For this review, take the finished solid that the model builds, in its own axes (mm). Give positions to 0.01 mm unless a question says otherwise; leave off trailing zeros. Write each loop counter-clockwise with the first axis right and the second up, starting at its lowest first coordinate (ties: lowest second). Pieces come first, ordered by that corner, then holes. Notation, with made-up numbers: M 48,-26 L 99,-26 A14 cw 99,-18 Z; hole C 5,84 d8. An arc over 180 degrees is marked long. Write item = value, one per line.
```python
from build123d import *

# Parameters (mm, degrees)
SKETCH1_R                  = 11.25
BOSS_EXTRUDE1_DEPTH        = 2.5
SKETCH2_R                  = 1.6
CUT_EXTRUDE1_DEPTH         = 2.5
M3_TAPPED_HOLE1_AT_2_COUNT = 2
M3_TAPPED_HOLE1_AT_2_PITCH = 32.526911935
CHAMFER1_SIZE              = 0.3


with BuildPart() as part:
    # Sketch1 → Boss-Extrude1 (new body)
    with BuildSketch(Plane.XY):
        Polygon((-14, -12.5), (-12.5, -14), (12.5, -14), (14, -12.5), (14, 12.5), (12.5, 14), (-12.5, 14), (-14, 12.5), align=None)
        Circle(SKETCH1_R, mode=Mode.SUBTRACT)
    extrude(amount=BOSS_EXTRUDE1_DEPTH)

    # Sketch2 → Cut-Extrude1 (cut)
    with BuildSketch(Plane.XY.offset(2.5)):
        with Locations((-11.5, 11.5)):
            Circle(SKETCH2_R)
        with Locations((11.5, -11.5)):
            Circle(SKETCH2_R)
    extrude(amount=-CUT_EXTRUDE1_DEPTH, mode=Mode.SUBTRACT)

    # Sketch4 → M3 Tapped Hole1 (revolve, cut)
    with BuildSketch(Plane(origin=(-11.5, -11.5, 2.5), x_dir=(0, -1, 0), z_dir=(1, 0, 0))):
        Polygon((0, 0), (0, 2.5), (1.6, 2.5), (1.25, 2.15), (1.25, 0.35), (1.6, 0), align=None)
    m3_tapped_hole1 = revolve(axis=Axis((-11.5, -11.5, 8.85), (0, 0, -1)), mode=Mode.SUBTRACT)

    # M3 Tapped Hole1 at 2: M3 Tapped Hole1 ×2
    with Locations(*[Vector(0.7071067811865476, 0.7071067811865476, 0) * (i * M3_TAPPED_HOLE1_AT_2_PITCH) for i in range(1, M3_TAPPED_HOLE1_AT_2_COUNT)]):
        add(m3_tapped_hole1, mode=Mode.SUBTRACT)

    # Chamfer1
    chamfer1_edges = [part.edges().sort_by_distance(p)[0] for p in [
        (13.25, -13.25, 0),
        (0, -14, 0),
        (-13.25, -13.25, 0),
        (-14, 0, 0),
        (0, -14, 2.5),
        (13.25, -13.25, 2.5),
        (14, 0, 2.5),
        (-11.25, 0, 0),
        (-11.25, 0, 2.5),
        (13.25, 13.25, 2.5),
        (0, 14, 2.5),
        (-13.1, 11.5, 0),
        (-13.1, 11.5, 2.5),
        (-13.25, 13.25, 2.5),
        (9.9, -11.5, 0),
        (9.9, -11.5, 2.5),
        (-14, 0, 2.5),
        (-13.25, 13.25, 0),
        (-13.25, -13.25, 2.5),
        (0, 14, 0),
        (13.25, 13.25, 0),
        (14, 0, 0),
    ]]
    chamfer(chamfer1_edges, length=CHAMFER1_SIZE)


solid = part.part
```
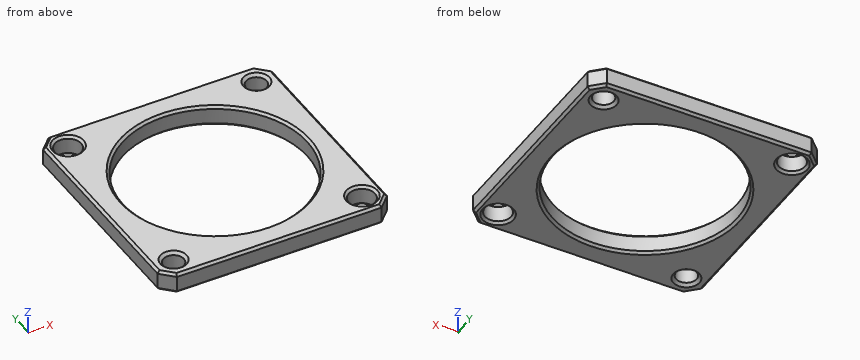
1. We need section B-B, the plane z = 1.4. Write out the cut boundary in (x, y).
Responses:
outline = M -14,-12.5 L -12.5,-14 L 12.5,-14 L 14,-12.5 L 14,12.5 L 12.5,14 L -12.5,14 L -14,12.5 Z; hole C -11.5,11.5 d3.2; hole C -11.5,-11.5 d2.5; hole C 0,0 d22.5; hole C 11.5,-11.5 d3.2; hole C 11.5,11.5 d2.5
2. Insertion check: P1, Ø3.5, axis at x = -11.5, y = 11.5, coming from the +Z side; P2, Ø1, axis at x = -10, y = 1.5, coming from the +Z side; P3, Ø1, axis at x = 10.5, y = -3, coming from the -Z side. Each pin has a flat end and moves straight along its axis. Give the tip position at first contact, or say it passes through.
Responses:
P1 = 2.35
P2 = through
P3 = 0.13
3. We need section A-A, the plane x = 0. Write out the cut boundary in (y, z), then the cut area to 3 significant figures.
Responses:
outline = M -14,0.3 L -13.7,0 L -11.55,0 L -11.25,0.3 L -11.25,2.2 L -11.55,2.5 L -13.7,2.5 L -14,2.2 Z; M 11.25,0.3 L 11.55,0 L 13.7,0 L 14,0.3 L 14,2.2 L 13.7,2.5 L 11.55,2.5 L 11.25,2.2 Z
area = 13.4 mm2
4. For line 1 along Y through (x, z) = (-11.5, 1.75); line 2 along Y through (x, z) = (0, 0.7); line 3 along Y through (x, z) = (-1.5, 1.55), list the stretches that pass through material, from the lowest coordinate up. Write a range as from..to.
Responses:
line_1 = -14..-12.75, -10.25..9.9, 13.1..14
line_2 = -14..-11.25, 11.25..14
line_3 = -14..-11.15, 11.15..14
5. We need section C-C, the plane x = -10.75. Count the separate pieces of the cut face and the enclosed holes in it, then the cut area to 3 significant figures.
Responses:
separate_pieces = 4
enclosed_holes = 0
area = 40.1 mm2
